Part print with two shaded views. Sizes in mm from the minimum x, y, z corner. A direction names the side the tool comes from. Give positions to 0.01 mm unless a question says otherwise; leave off trailing zeros. Order: outer loops, then holes, each group sorted by start corner. A loop starts at its lowest first (then second) coordinate and runs counter-clockwise, first axis right, second up. Notation, with made-up numbers: (65.5, 8.5) -> (124.5, 8.5) arc R21 cw to (124.5, 40.5) -> close; hole circle Ø4 at (-23, 39.5). An arc over 180 degrees is marked (long way). Write item = value, one per line. Start each with the question number.
Item 1: Flat gauge pins, fed straight in: P1, Ø15, axis at x = 581, z = 185.5, coming from the -Y side; P2, Ø15, axis at x = 460.5, z = 124.5, coming from the -Y side; P3, Ø4, axis at x = 691, z = 524, coming from the -Y side. Where does each tip first touch, or does it go through?
Item 2: Pull direction X, two halves, no side cores. Call the marked faces 6, 7 and 8: +X half, -X half, draft (parallel to the pull), parting line (faces both ways), or undercut.
Item 3: Drill centre lines: line 1 along X through (y, z) = (370, 404); line 2 along Z through (x, y) = (152, 496); line 3 along Y through (x, z) = (752, 632). Where is each one in solid material? Low to high.
Item 4: Tool access for the marked faces 1, 2, 3, 4 and 5: list every direction of +Z, -Z, +X, -X, +Y, -Y with a clear straight run to the whole face (end or side of a thin tool).
Item 5: Band-saw the part on B-B on x = 723.5. Write the cut outline in (y, z), plus the area to 3 significant figures.
Item 6: Band-saw the part on C-C on z = 121.5. Write the cut outline in (x, y).
Item 7: Band-saw the part on D-D on x = 400.5. Write the cut outline in (y, z), plus the area to 3 significant figures.
Item 8: Band-saw the part on A-A on y = 490.5. Write the cut outline in (x, z).
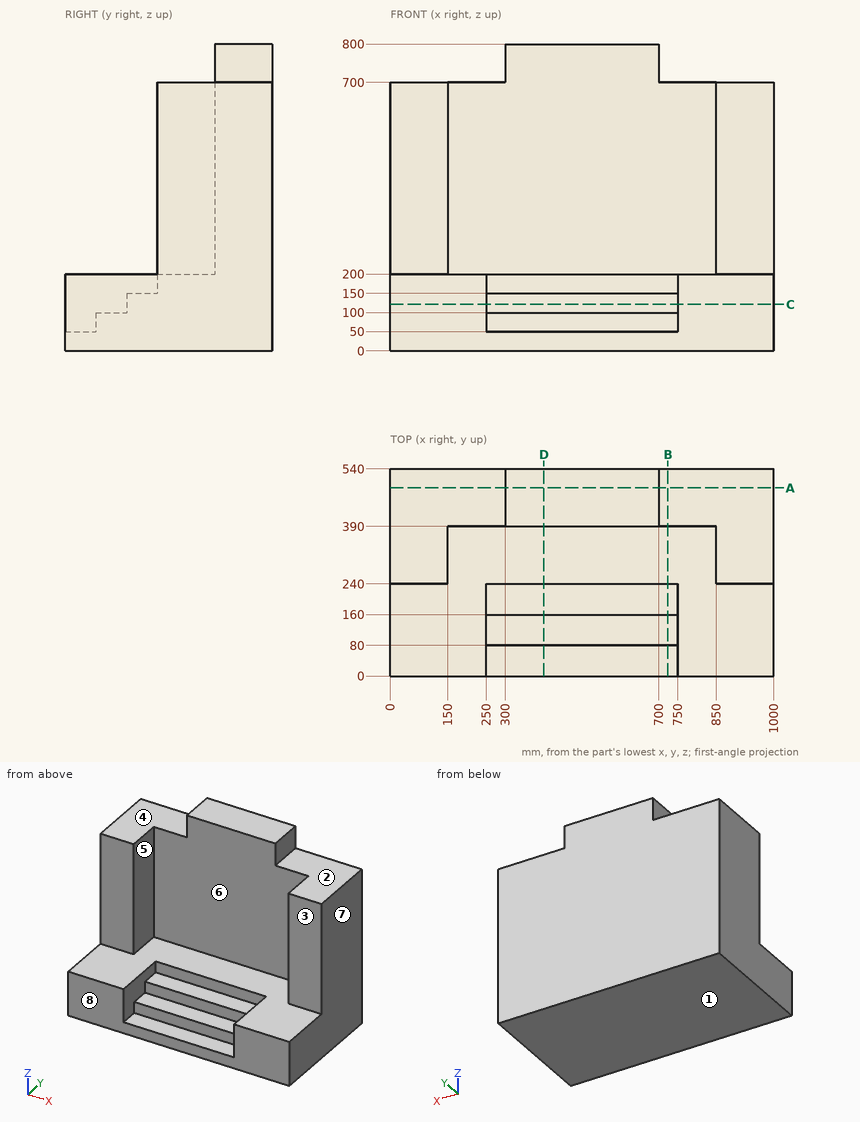
Values found:
q1.P1 = 240
q1.P2 = 160
q1.P3 = 390
q2.face_6 = undercut
q2.face_7 = +X half
q2.face_8 = draft
q3.line_1 = 0 to 150, 850 to 1000
q3.line_2 = 0 to 700
q3.line_3 = 390 to 540
q4.face_1 = -Z, +X, -X, +Y, -Y
q4.face_2 = +Z, +X, +Y, -Y
q4.face_3 = +Z, +X, -X, -Y
q4.face_4 = +Z, -X, +Y, -Y
q4.face_5 = +Z, -Y
q5.outline = (0, 0) -> (540, 0) -> (540, 700) -> (390, 700) -> (390, 200) -> (240, 200) -> (240, 150) -> (160, 150) -> (160, 100) -> (80, 100) -> (80, 50) -> (0, 50) -> close
q5.area = 159,000 mm^2
q6.outline = (0, 0) -> (250, 0) -> (250, 160) -> (750, 160) -> (750, 0) -> (1000, 0) -> (1000, 540) -> (0, 540) -> close
q7.outline = (0, 0) -> (540, 0) -> (540, 800) -> (390, 800) -> (390, 200) -> (240, 200) -> (240, 150) -> (160, 150) -> (160, 100) -> (80, 100) -> (80, 50) -> (0, 50) -> close
q7.area = 174,000 mm^2
q8.outline = (0, 0) -> (1000, 0) -> (1000, 700) -> (700, 700) -> (700, 800) -> (300, 800) -> (300, 700) -> (0, 700) -> close
